from build123d import *

# Parameters (mm, degrees)
BEND_BODY_DEPTH               = 55
BEND_BODY_2_DEPTH             = 55
FLANGE_A_SKETCH_W             = 24
FLANGE_A_SKETCH_H             = 13
FLANGE_A_DEPTH                = 5
FLANGE_B_SKETCH_W             = 13
FLANGE_B_SKETCH_H             = 24
FLANGE_B_DEPTH                = 5
FLANGE_START                  = -15
FLANGE_B_TRANSITION_CUT_DEPTH = 15
FLANGE_A_TRANSITION_CUT_DEPTH = 15
FLANGE_START_2                = 2
FLANGE_A_PAD_1_DEPTH          = 2
FLANGE_B_PAD_1_DEPTH          = 2
FLANGE_B_PAD_2_DEPTH          = 2
FLANGE_START_3                = -2
FLANGE_B_PAD_3_DEPTH          = 2
FLANGE_A_PAD_2_DEPTH          = 2
FLANGE_A_PAD_3_DEPTH          = 2
FLANGE_A_PAD_4_DEPTH          = 2
BOLT_HOLES_SET_1_SKETCH_R     = 3
BOLT_HOLES_SET_1_4X_DEPTH     = 5
BOLT_HOLES_SET_2_SKETCH_R     = 3
BOLT_HOLES_SET_2_4X_DEPTH     = 5


with BuildPart() as part:
    # Bend Profile Sketch → Bend Body (new body)
    with BuildSketch(Plane.XY):
        with BuildLine():
            Line((0, 57), (-5, 57))
            Line((-5, 57), (-5, 70))
            Line((-5, 70), (0, 70))
            Line((0, 70), (0, 60))
            ThreePointArc((0, 60), (42.426406871, 42.426406871), (60, 0))
            Line((60, 0), (70, 0))
            Line((70, 0), (70, -5))
            Line((70, -5), (57, -5))
            Line((57, -5), (57, 0))
            ThreePointArc((57, 0), (40.305086528, 40.305086528), (0, 57))
        make_face()
    extrude(amount=BEND_BODY_DEPTH)



with BuildPart() as body_2:
    # Bend Profile Sketch → Bend Body 2 (new body)
    with BuildSketch(Plane.XY):
        with BuildLine():
            Line((0, 33), (-5, 33))
            Line((-5, 33), (-5, 20))
            Line((-5, 20), (0, 20))
            Line((0, 20), (0, 30))
            ThreePointArc((0, 30), (21.213203436, 21.213203436), (30, 0))
            Line((30, 0), (20, 0))
            Line((20, 0), (20, -5))
            Line((20, -5), (33, -5))
            Line((33, -5), (33, 0))
            ThreePointArc((33, 0), (23.334523779, 23.334523779), (0, 33))
        make_face()
    extrude(amount=BEND_BODY_2_DEPTH)


with BuildPart() as part_1:
    add(part.part)

    add(body_2.part)  # Flange A merges body 2
    # Flange A Sketch → Flange A (add)
    with BuildSketch(Plane(origin=(0, -5, 0), x_dir=(-1, 0, 0), z_dir=(0, -1, 0))):
        with Locations((-45, -48.5)):
            Rectangle(FLANGE_A_SKETCH_W, FLANGE_A_SKETCH_H)
        with Locations((-45, -6.5)):
            Rectangle(FLANGE_A_SKETCH_W, FLANGE_A_SKETCH_H)
    extrude(amount=-FLANGE_A_DEPTH)

    # Flange B Sketch → Flange B (add)
    with BuildSketch(Plane.ZY.offset(5)):
        with Locations((48.5, 45)):
            Rectangle(FLANGE_B_SKETCH_W, FLANGE_B_SKETCH_H)
        with Locations((6.5, 45)):
            Rectangle(FLANGE_B_SKETCH_W, FLANGE_B_SKETCH_H)
    extrude(amount=-FLANGE_B_DEPTH)

    # Flange B Transition Cut Sketch → Flange B Transition Cut (cut)
    with BuildSketch(Plane.XY.offset(55).offset(FLANGE_START)):
        with BuildLine():
            Line((57, 0), (60, 0))
            ThreePointArc((60, 0), (42.426406871, 42.426406871), (0, 60))
            Line((0, 60), (0, 57))
            ThreePointArc((0, 57), (40.305086528, 40.305086528), (57, 0))
        make_face()
        with BuildLine():
            Line((30, 0), (33, 0))
            ThreePointArc((33, 0), (23.334523779, 23.334523779), (0, 33))
            Line((0, 33), (0, 30))
            ThreePointArc((0, 30), (21.213203436, 21.213203436), (30, 0))
        make_face()
    extrude(amount=FLANGE_B_TRANSITION_CUT_DEPTH, mode=Mode.SUBTRACT)

    # Flange A Transition Cut Sketch → Flange A Transition Cut (cut)
    with BuildSketch(Plane(origin=(0, 0, 0), x_dir=(-1, 0, 0), z_dir=(0, 0, -1))):
        with BuildLine():
            Line((0, 57), (0, 60))
            ThreePointArc((0, 60), (-42.426406871, 42.426406871), (-60, 0))
            Line((-60, 0), (-57, 0))
            ThreePointArc((-57, 0), (-40.305086528, 40.305086528), (0, 57))
        make_face()
        with BuildLine():
            Line((0, 30), (0, 33))
            ThreePointArc((0, 33), (-23.334523779, 23.334523779), (-33, 0))
            Line((-33, 0), (-30, 0))
            ThreePointArc((-30, 0), (-21.213203436, 21.213203436), (0, 30))
        make_face()
    extrude(amount=-FLANGE_A_TRANSITION_CUT_DEPTH, mode=Mode.SUBTRACT)

    # Flange A Pad 1 Sketch → Flange A Pad 1 (add)
    with BuildSketch(Plane(origin=(0, 0, 15), x_dir=(-1, 0, 0), z_dir=(0, 0, -1)).offset(FLANGE_START_2)):
        with BuildLine():
            Line((0, 60), (0, 57))
            ThreePointArc((0, 57), (-40.305086528, 40.305086528), (-57, 0))
            Line((-57, 0), (-60, 0))
            ThreePointArc((-60, 0), (-42.426406871, 42.426406871), (0, 60))
        make_face()
        with BuildLine():
            Line((-33, 0), (-30, 0))
            ThreePointArc((-30, 0), (-21.213203436, 21.213203436), (0, 30))
            Line((0, 30), (0, 33))
            ThreePointArc((0, 33), (-23.334523779, 23.334523779), (-33, 0))
        make_face()
    extrude(amount=-FLANGE_A_PAD_1_DEPTH)

    # Flange B Pad 1 Sketch → Flange B Pad 1 (add)
    with BuildSketch(Plane.XY.offset(40)):
        with BuildLine():
            Line((0, 60), (0, 57))
            ThreePointArc((0, 57), (40.305086528, 40.305086528), (57, 0))
            Line((57, 0), (60, 0))
            ThreePointArc((60, 0), (42.426406871, 42.426406871), (0, 60))
        make_face()
        with BuildLine():
            Line((30, 0), (33, 0))
            ThreePointArc((33, 0), (23.334523779, 23.334523779), (0, 33))
            Line((0, 33), (0, 30))
            ThreePointArc((0, 30), (21.213203436, 21.213203436), (30, 0))
        make_face()
    extrude(amount=FLANGE_B_PAD_1_DEPTH)

    # Flange B Pad 2 Sketch → Flange B Pad 2 (add)
    with BuildSketch(Plane.XY.offset(42)):
        with BuildLine():
            Line((0, 60), (0, 57))
            ThreePointArc((0, 57), (40.305086528, 40.305086528), (57, 0))
            Line((57, 0), (60, 0))
            ThreePointArc((60, 0), (42.426406871, 42.426406871), (0, 60))
        make_face()
        with BuildLine():
            ThreePointArc((33, 0), (23.334523779, 23.334523779), (0, 33))
            Line((0, 33), (0, 30))
            ThreePointArc((0, 30), (21.213203436, 21.213203436), (30, 0))
            Line((30, 0), (33, 0))
        make_face()
    extrude(amount=FLANGE_B_PAD_2_DEPTH)

    # Flange B Pad 3 Sketch → Flange B Pad 3 (add)
    with BuildSketch(Plane.XY.offset(44).offset(FLANGE_START_3)):
        with BuildLine():
            ThreePointArc((57, 0), (40.305086528, 40.305086528), (0, 57))
            Line((0, 57), (0, 33))
            ThreePointArc((0, 33), (23.334523779, 23.334523779), (33, 0))
            Line((33, 0), (57, 0))
        make_face()
    extrude(amount=FLANGE_B_PAD_3_DEPTH)

    # Flange A Pad 2 Sketch → Flange A Pad 2 (add)
    with BuildSketch(Plane(origin=(0, 0, 13), x_dir=(-1, 0, 0), z_dir=(0, 0, -1)).offset(FLANGE_START_2)):
        with BuildLine():
            Line((0, 57), (0, 60))
            ThreePointArc((0, 60), (-42.426406871, 42.426406871), (-60, 0))
            Line((-60, 0), (-57, 0))
            ThreePointArc((-57, 0), (-40.305086528, 40.305086528), (0, 57))
        make_face()
        with BuildLine():
            Line((0, 30), (0, 33))
            ThreePointArc((0, 33), (-23.334523779, 23.334523779), (-33, 0))
            Line((-33, 0), (-30, 0))
            ThreePointArc((-30, 0), (-21.213203436, 21.213203436), (0, 30))
        make_face()
    extrude(amount=-FLANGE_A_PAD_2_DEPTH)

    # Flange A Pad 3 Sketch → Flange A Pad 3 (add)
    with BuildSketch(Plane(origin=(0, 0, 11), x_dir=(-1, 0, 0), z_dir=(0, 0, -1)).offset(FLANGE_START_2)):
        with BuildLine():
            Line((0, 57), (0, 60))
            ThreePointArc((0, 60), (-42.426406871, 42.426406871), (-60, 0))
            Line((-60, 0), (-57, 0))
            ThreePointArc((-57, 0), (-40.305086528, 40.305086528), (0, 57))
        make_face()
        with BuildLine():
            Line((0, 30), (0, 33))
            ThreePointArc((0, 33), (-23.334523779, 23.334523779), (-33, 0))
            Line((-33, 0), (-30, 0))
            ThreePointArc((-30, 0), (-21.213203436, 21.213203436), (0, 30))
        make_face()
    extrude(amount=-FLANGE_A_PAD_3_DEPTH)

    # Flange A Pad 4 Sketch → Flange A Pad 4 (add)
    with BuildSketch(Plane(origin=(0, 0, 9), x_dir=(-1, 0, 0), z_dir=(0, 0, -1))):
        with BuildLine():
            Line((-57, 0), (-33, 0))
            ThreePointArc((-33, 0), (-23.334523779, 23.334523779), (0, 33))
            Line((0, 33), (0, 57))
            ThreePointArc((0, 57), (-40.305086528, 40.305086528), (-57, 0))
        make_face()
    extrude(amount=-FLANGE_A_PAD_4_DEPTH)

    # Bolt Holes Set 1 Sketch → Bolt Holes Set 1 4x (cut)
    with BuildSketch(Plane.ZY.offset(5)):
        with Locations((6.5, 63.5)):
            Circle(BOLT_HOLES_SET_1_SKETCH_R)
        with Locations((48.5, 63.5)):
            Circle(BOLT_HOLES_SET_1_SKETCH_R)
        with Locations((48.5, 26.5)):
            Circle(BOLT_HOLES_SET_1_SKETCH_R)
        with Locations((6.5, 26.5)):
            Circle(BOLT_HOLES_SET_1_SKETCH_R)
    extrude(amount=-BOLT_HOLES_SET_1_4X_DEPTH, mode=Mode.SUBTRACT)

    # Bolt Holes Set 2 Sketch → Bolt Holes Set 2 4x (cut)
    with BuildSketch(Plane.XZ.offset(5)):
        with Locations(Location((26.5, 48.5, 0), (0, 0, 270))):
            Circle(BOLT_HOLES_SET_2_SKETCH_R)
        with Locations(Location((63.5, 48.5, 0), (0, 0, 270))):
            Circle(BOLT_HOLES_SET_2_SKETCH_R)
        with Locations(Location((63.5, 6.5, 0), (0, 0, 270))):
            Circle(BOLT_HOLES_SET_2_SKETCH_R)
        with Locations(Location((26.5, 6.5, 0), (0, 0, 270))):
            Circle(BOLT_HOLES_SET_2_SKETCH_R)
    extrude(amount=-BOLT_HOLES_SET_2_4X_DEPTH, mode=Mode.SUBTRACT)


solid = part_1.part
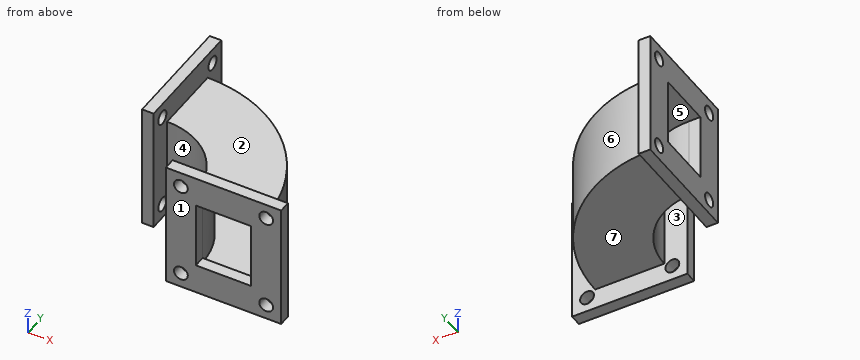
Part model, mm, in its own coordinate system. Face numbers are marked on the shaded views. A direction names the side the tool comes from. Coordinates: 2 decimals unless noted, no trailing zeros. Order: outer loops, then holes, each group sorted by start corner. A loop starts at its lowest first (then second) coordinate and runs counter-clockwise, first axis right, second up.
(1) Pin check, flat tips, straight feed: pin 1 Ø1.5 at (x, y) = (59, 19) entering from -Z; pin 2 Ø1.6 at (x, z) = (42, 12.5) entering from +Y; pin 3 Ø1.5 at (x, y) = (40.5, 15) entering from -Z; pin 4 Ø5.5 at (y, z) = (-1.5, 30.5) entering from -X. Stop position of each tip, or through.
Check sheet entries:
pin 1: passes through
pin 2: stops at y = 43.62
pin 3: stops at z = 9
pin 4: stops at x = 20
(2) Pull direction Y, two halves, no side cores. Call the marked faces 1, 2 and 3: pulls with the +Y half, pulls with the -Y half, needs draft (parallel to the pull), parting line crosses it, or undercut.
Check sheet entries:
face 1: pulls with the -Y half
face 2: needs draft
face 3: undercut
(3) Slice it at D-D, the plane z = 14.5. Write the cut outline in (x, y), and give its area (3 significant figures).
Check sheet entries:
outline: (-5, 20) - (0, 20) - (0, 30) arc R30 cw to (30, 0) - (20, 0) - (20, -5) - (33, -5) - (33, 0) arc R33 ccw to (0, 33) - (-5, 33) - close; (-5, 57) - (0, 57) arc R57 cw to (57, 0) - (57, -5) - (70, -5) - (70, 0) - (60, 0) arc R60 ccw to (0, 60) - (0, 70) - (-5, 70) - close
area: 684 mm2
(4) Slice it at A-A, the plane z = 6.5. Write the cut outline in (x, y).
Check sheet entries:
outline: (-5, 20) - (0, 20) - (0, 23.5) - (-5, 23.5) - close; (-5, 29.5) - (0, 29.5) - (0, 60.5) - (-5, 60.5) - close; (-5, 66.5) - (0, 66.5) - (0, 70) - (-5, 70) - close; (20, -5) - (23.5, -5) - (23.5, 0) - (20, 0) - close; (29.5, -5) - (60.5, -5) - (60.5, 0) - (29.5, 0) - close; (66.5, -5) - (70, -5) - (70, 0) - (66.5, 0) - close
(5) Slice it at C-C, the plane x = 27.5. Write the cut outline in (y, z), and give its area (3 significant figures).
Check sheet entries:
outline: (-5, 0) - (0, 0) - (0, 3.67) - (-5, 3.67) - close; (-5, 9.33) - (0, 9.33) - (0, 45.67) - (-5, 45.67) - close; (-5, 51.33) - (0, 51.33) - (0, 55) - (-5, 55) - close; (11.99, 9) - (53.33, 9) - (53.33, 44) - (11.99, 44) - close; hole (18.24, 11) - (49.93, 11) - (49.93, 42) - (18.24, 42) - close
area: 683 mm2
(6) Tool access for the marked faces 4, 5, 6 and 7: list every direction of +Z, -Z, +X, -X, +Y, -Y with a clear straight run to the whole face (end or side of a thin tool).
Check sheet entries:
face 4: +Z, -Z
face 5: none
face 6: +Z, -Z, +X, +Y
face 7: -Z, +X, +Y
(7) Slice it at B-B, the plane y = 24.5. Write the cut outline in (x, z).
Check sheet entries:
outline: (-5, 0) - (0, 0) - (0, 4.26) - (-5, 4.26) - close; (-5, 8.74) - (0, 8.74) - (0, 46.26) - (-5, 46.26) - close; (-5, 50.74) - (0, 50.74) - (0, 55) - (-5, 55) - close; (17.31, 9) - (54.77, 9) - (54.77, 44) - (17.31, 44) - close; hole (22.11, 11) - (51.47, 11) - (51.47, 42) - (22.11, 42) - close
(8) Probe L1, parallel to Y at x = -1.35, z = 48.5; L2, parallel to Z at x = 63, y = -1. List the from-to ranges inside material, lowest first.
Check sheet entries:
L1: y = 20 to 23.5, 29.5 to 60.5, 66.5 to 70
L2: z = 0 to 3.54, 9.46 to 45.54, 51.46 to 55
